Design review of the part built by this model. Coordinates are the model's own, in mm. Face numbers are marked on the shaded views. A direction names the side the tool comes from. Coordinates: 2 decimals unless noted, no trailing zeros. Loops run counter-clockwise (first coordinate to the right, second up) from the corner with the lowest first, then second, coordinate; pieces in that order, holes last. Notation, with made-up numbers: (12.5, 7) -> (31.5, 7) arc R19 ccw to (31.5, 19) -> close; hole circle Ø3 at (47, -2.75). An arc over 180 degrees is marked (long way). Answer as a JSON object with one key per item and string values.
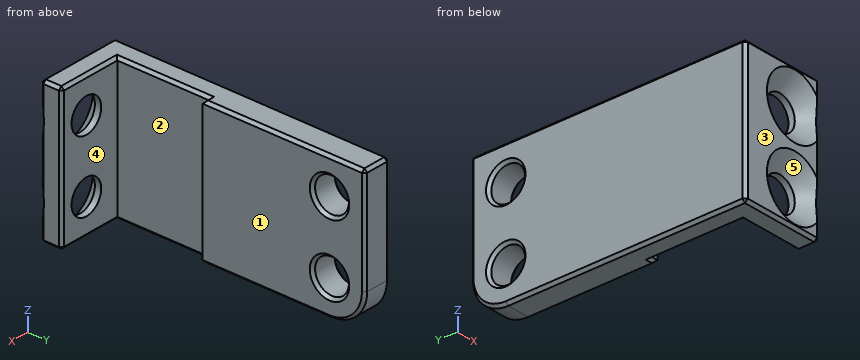
```python
from build123d import *

# Parameters (mm, degrees)
SKETCH1_W                                    = 2
SKETCH1_H                                    = 10
BOSS_EXTRUDE1_DEPTH                          = 19.5
SKETCH2_R                                    = 1.2
CUT_EXTRUDE1_DEPTH                           = 20
SKETCH3_W                                    = 10
SKETCH3_H                                    = 1.5
BOSS_EXTRUDE2_DEPTH                          = 4
SKETCH4_W                                    = 10
SKETCH4_H                                    = 6.5
CUT_EXTRUDE2_DEPTH                           = 0.5
HOLE_SIZE_SLOTTED_COUNTERSUNK_WOOD_S_2_COUNT = 2
HOLE_SIZE_SLOTTED_COUNTERSUNK_WOOD_S_2_PITCH = 5
FILLET1_R                                    = 2.5
CHAMFER1_SIZE                                = 0.2


with BuildPart() as part:
    # Sketch1 → Boss-Extrude1 (new body)
    with BuildSketch(Plane(origin=(0, 0, 0), x_dir=(1, 0, 0), z_dir=(0, 1, 0))):
        with Locations((1, 5)):
            Rectangle(SKETCH1_W, SKETCH1_H)
    extrude(amount=BOSS_EXTRUDE1_DEPTH)

    # Sketch2 → Cut-Extrude1 (cut)
    with BuildSketch(Plane(origin=(2, 0, 0), x_dir=(0, 0, -1), z_dir=(1, 0, 0))):
        with Locations((2.5, 17)):
            Circle(SKETCH2_R)
        with Locations((7.5, 17)):
            Circle(SKETCH2_R)
    extrude(amount=-CUT_EXTRUDE1_DEPTH, mode=Mode.SUBTRACT)

    # Sketch3 → Boss-Extrude2 (add)
    with BuildSketch(Plane(origin=(2, 0, 0), x_dir=(0, 0, -1), z_dir=(1, 0, 0))):
        with Locations((5, 0.75)):
            Rectangle(SKETCH3_W, SKETCH3_H)
    extrude(amount=BOSS_EXTRUDE2_DEPTH)

    # Sketch4 → Cut-Extrude2 (cut)
    with BuildSketch(Plane(origin=(2, 0, 0), x_dir=(0, 0, -1), z_dir=(1, 0, 0))):
        with Locations((5, 4.75)):
            Rectangle(SKETCH4_W, SKETCH4_H)
    extrude(amount=-CUT_EXTRUDE2_DEPTH, mode=Mode.SUBTRACT)

    # Sketch6 → Hole size slotted countersunk wood screw type 0 (revolve, cut)
    with BuildSketch(Plane(origin=(4, 0, -2.5), x_dir=(0, 0, -1), z_dir=(1, 0, 0))):
        Polygon((0, 0), (0, 1.5), (1.2, 1.5), (1.2, 1.05), (2.25, 0), align=None)
    hole_size_slotted_countersunk_wood_screw = revolve(axis=Axis((4, -6.35, -2.5), (0, 1, 0)), mode=Mode.SUBTRACT)

    # Hole size slotted countersunk wood s 2: Hole size slotted countersunk wood screw type 0 ×2
    with Locations(*[(0, 0, -i * HOLE_SIZE_SLOTTED_COUNTERSUNK_WOOD_S_2_PITCH) for i in range(1, HOLE_SIZE_SLOTTED_COUNTERSUNK_WOOD_S_2_COUNT)]):
        add(hole_size_slotted_countersunk_wood_screw, mode=Mode.SUBTRACT)

    # Fillet1
    fillet1_edges = [part.edges().sort_by_distance(p)[0] for p in [
        (1, 19.5, -10),
    ]]
    fillet(fillet1_edges, radius=FILLET1_R)

    # Chamfer1
    chamfer1_edges = [part.edges().sort_by_distance(p)[0] for p in [
        (0, 17, -6.3),
        (0, 17, -1.3),
        (6, 0, -5),
        (2, 19.5, -3.75),
        (2, 18.767766953, -9.267766953),
        (3, 0, -10),
        (6, 0, -9.265388203),
        (6, 0.75, -10),
        (2, 12.5, -10),
        (1.75, 8, -10),
        (1.5, 4.75, -10),
        (3.75, 1.5, -10),
        (3.75, 1.5, 0),
        (1.5, 4.75, 0),
        (1.75, 8, 0),
        (2, 13.75, 0),
        (1, 19.5, 0),
        (0, 9.75, 0),
        (0, 19.5, -3.75),
        (0, 18.767766953, -9.267766953),
        (0, 8.5, -10),
        (0, 0, -5),
        (3, 0, 0),
        (6, 0, -0.734611797),
        (6, 0.75, 0),
        (6, 1.5, -5),
        (2, 17, -1.3),
        (2, 17, -6.3),
    ]]
    chamfer(chamfer1_edges, length=CHAMFER1_SIZE)


solid = part.part
```
1) Wall thickness on probe 1 along Z at (x, y) = (4, 1.2); probe 2 along X at (y, z) = (8.25, -6.5); probe 3 along Z at (x, y) = (3.5, 1.25): over which ranges is each line inside the solid? List them lowest first.
Completed:
{"probe 1": "-10 to -8.7, -6.3 to -3.7, -1.3 to 0", "probe 2": "0 to 2", "probe 3": "-10 to -8.59, -6.41 to -3.59, -1.41 to 0"}
2) Clearance check with flat-ended pins moving along their axes: pin 1 Ø3 at (x, z) = (4, -7.5) entering from -Y; pin 2 Ø3 at (y, z) = (6, -3.5) entering from +X. State where each tip first meets the part, or that it passes through.
Completed:
{"pin 1": "y = 0.75", "pin 2": "x = 1.5"}
3) Add section C-C, the plane x = 4. Give the boundary of the cut face in (y, z).
Completed:
{"outline": "(0, -9.8) -> (0.2, -10) -> (1.3, -10) -> (1.5, -9.8) -> (1.5, -8.7) -> (1.05, -8.7) -> (0, -9.75) -> close; (0, -5.25) -> (1.05, -6.3) -> (1.5, -6.3) -> (1.5, -3.7) -> (1.05, -3.7) -> (0, -4.75) -> close; (0, -0.25) -> (1.05, -1.3) -> (1.5, -1.3) -> (1.5, -0.2) -> (1.3, 0) -> (0.2, 0) -> (0, -0.2) -> close"}
4) For the marked faces 4 and 5, list the 3-axis set-ups (+Z, -Z, +X, -X, +Y, -Y) from which the entire face can be reached by the end or side of a thin tool; tool diameter is ignored.
Completed:
{"face 4": "+Z, -Z, +X", "face 5": "-Y"}
5) Add section A-A, the plane x = 0.75. Give the boundary of the cut face in (y, z).
Completed:
{"outline": "(0, -9.8) -> (0.2, -10) -> (17, -10) arc R2.5 ccw to (19.5, -7.5) -> (19.5, -0.2) -> (19.3, 0) -> (0.2, 0) -> (0, -0.2) -> close; hole circle Ø2.4 at (17, -7.5); hole circle Ø2.4 at (17, -2.5)"}
6) Add section D-D, the plane y = 12. Give the boundary of the cut face in (x, z), and give its area (3 significant figures).
Completed:
{"outline": "(0, -9.8) -> (0.2, -10) -> (1.8, -10) -> (2, -9.8) -> (2, -0.2) -> (1.8, 0) -> (0.2, 0) -> (0, -0.2) -> close", "area": "19.9 mm²"}
7) Add section B-B, the plane z = -2.5. Give the boundary of the cut face in (x, y), and give its area (3 significant figures).
Completed:
{"outline": "(0, 0.2) -> (0.2, 0) -> (1.75, 0) -> (2.8, 1.05) -> (2.8, 1.5) -> (1.5, 1.5) -> (1.5, 8) -> (2, 8) -> (2, 15.6) -> (1.8, 15.8) -> (0.2, 15.8) -> (0, 15.6) -> close; (0, 18.4) -> (0.2, 18.2) -> (1.8, 18.2) -> (2, 18.4) -> (2, 19.3) -> (1.8, 19.5) -> (0.2, 19.5) -> (0, 19.3) -> close; (5.2, 1.05) -> (6, 0.25) -> (6, 1.3) -> (5.8, 1.5) -> (5.2, 1.5) -> close", "area": "32.1 mm²"}
8) The part is to be moulded in two halves that separate along Y. For the marked faces 1, 2 and 3, say which applies: pulls with the +Y half, pulls with the -Y half, needs draft (parallel to the pull), parting line crosses it, or undercut.
Completed:
{"face 1": "needs draft", "face 2": "undercut", "face 3": "pulls with the -Y half"}
